Verification items for the finished model (mm, model axes). Face numbers are marked on the shaded views. Round coordinates to 2 decimals unless told otherwise and drop trailing zeros. Loops run counter-clockwise (first coordinate to the right, second up) from the corner with the lowest first, then second, coordinate; pieces in that order, holes last.
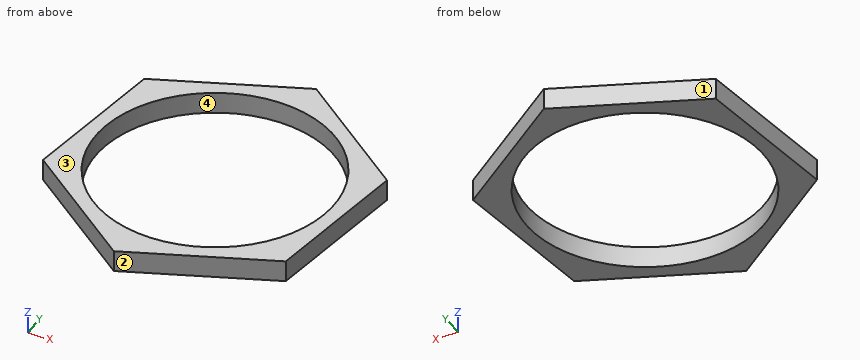
from build123d import *

# Parameters (mm, degrees)
SKETCH_1_R      = 11
EXTRUDE_1_DEPTH = 2


with BuildPart() as part:
    # 草图1 → 凸台-拉伸1 (new body)
    with BuildSketch(Plane.XY):
        Polygon((9.893192504, 17.474140349), (11.633566446, 31.61746381), (0.255276005, 40.196333587), (-12.863388378, 34.631879902), (-14.60376232, 20.48855644), (-3.225471879, 11.909686664), align=None)
        with Locations((-1.485097937, 26.053010125)):
            Circle(SKETCH_1_R, mode=Mode.SUBTRACT)
    extrude(amount=EXTRUDE_1_DEPTH)


solid = part.part
1. Section check A-A (y = 30). Enter the section's corners in (x, z), then the cut area to 3 significant figures.
2. Section check C-C (z = 1.4). Enter the section's corners in (x, y).
3. Release check for a two-part mould opening along Y. For the marked faces 1, 2, 3 and 4 record: released by +Y, released by -Y, zero draft, split by the parting line, or undercut.
4. Scan lines: L1, parallel to X at y = 34, z = 1.8; L2, parallel to X at y = 17.25, z = 0.3; L3, parallel to Y at x = 1.5, z = 0.7. Record each from-to range of solid material in increasing order.
5. Section check B-B (x = 5.5). Enter the section's corners in (y, z), then the cut area to 3 significant figures.
Taken from the geometry:
1. outline: (-13.43, 0) - (-11.75, 0) - (-11.75, 2) - (-13.43, 2) - close; (8.78, 0) - (11.43, 0) - (11.43, 2) - (8.78, 2) - close
1. area: 8.67 mm2
2. outline: (-14.6, 20.49) - (-3.23, 11.91) - (9.89, 17.47) - (11.63, 31.62) - (0.26, 40.2) - (-12.86, 34.63) - close; hole circle Ø22 at (-1.49, 26.05)
3. face 1: released by +Y
3. face 2: released by -Y
3. face 3: zero draft
3. face 4: undercut
4. L1: x = -12.94 to -9.09, 6.12 to 8.47
4. L2: x = -10.31 to -8.08, 5.11 to 9.36
4. L3: y = 13.91 to 15.47, 36.64 to 39.26
5. outline: (15.61, 0) - (17.56, 0) - (17.56, 2) - (15.61, 2) - close; (34.55, 0) - (36.24, 0) - (36.24, 2) - (34.55, 2) - close
5. area: 7.27 mm2
